Geometry: see drawing. Coordinates: mm, zero at the bounding-box minimum. A direction names the side the tool comes from. Round coordinates to 2 decimals unless told otherwise and drop trailing zeros. Loops run counter-clockwise (first coordinate to the right, second up) from the corner with the lowest first, then second, coordinate; pieces in that order, holes last.
(1) Draft query along Y for the marked faces 5, 6, 7 and 8. Return one class per face: released by +Y, released by -Y, zero draft, split by the parting line, or undercut.
(2) First-contact query: pin 1 Ø4 at (x, y) = (115, 1058.5) entering from +Z; pin 2 Ø2 at (y, z) = (1742, 258) entering from +X; pin 3 Ø10 at (x, y) = (319, 1799.5) entering from -Z. Flat tips, straight axial feed; report the tip coordinate or a pass-through.
(3) Access query for the marked faces 1, 2, 3 and 4. Directions: +Z, -Z, +X, -X, +Y, -Y. A direction counts if a zero-diameter tool reaches every point of the face in a straight line with its end or side. Return the directions, or none.
(4) Cut plane A-A, the plane z = 303. Output: boundary loops of the cut face in (x, y).
(5) Cut plane D-D, the plane z = 72. Output: boundary loops of the cut face in (x, y).
(6) Cut plane B-B, the plane x = 272. Output: boundary loops of the cut face in (y, z), and give its area (4 significant figures).
(7) Line query: line 1 (Z direction, x = 288.5, y = 1199.5); line 2 (Z direction, x = 325, y = 2006.5); line 3 (X direction, y = 1922, z = 234.5). Output: solid intervals per line, ascending.
(8) Cut plane C-C, the plane y = 1827. Output: boundary loops of the cut face in (x, z), and give its area (3 significant figures).
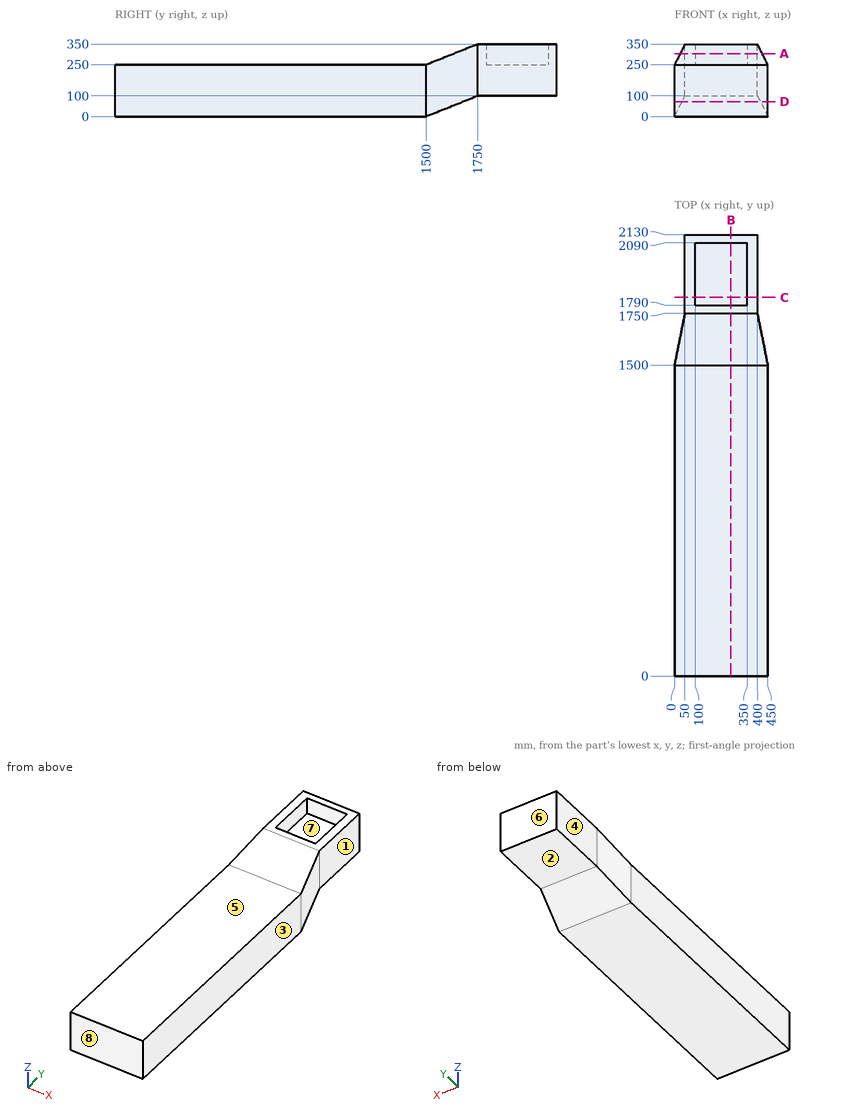
Reported:
1. face 5: zero draft
1. face 6: released by +Y
1. face 7: undercut
1. face 8: released by -Y
2. pin 1: stops at z = 250
2. pin 2: stops at x = 401.8
2. pin 3: stops at z = 100
3. face 1: +Z, -Z, +X, +Y
3. face 2: -Z, +X, -X, +Y
3. face 3: +Z, -Z, +X, +Y, -Y
3. face 4: +Z, -Z, -X, +Y
4. outline: (26.5, 1632.5) - (423.5, 1632.5) - (400, 1750) - (400, 2130) - (50, 2130) - (50, 1750) - close; hole (100, 1790) - (350, 1790) - (350, 2090) - (100, 2090) - close
5. outline: (0, 0) - (450, 0) - (450, 1500) - (414, 1680) - (36, 1680) - (0, 1500) - close
6. outline: (0, 0) - (1500, 0) - (1750, 100) - (2130, 100) - (2130, 350) - (2090, 350) - (2090, 250) - (1790, 250) - (1790, 350) - (1750, 350) - (1500, 250) - (0, 250) - close
6. area: 502,500 mm2
7. line 1: z = 0 to 250
7. line 2: z = 100 to 250
7. line 3: x = 50 to 400
8. outline: (50, 100) - (400, 100) - (400, 350) - (350, 350) - (350, 250) - (100, 250) - (100, 350) - (50, 350) - close
8. area: 62,500 mm2
